Design review of the part built by this model. Coordinates are the model's own, in mm. A direction names the side the tool comes from. Coordinates: 2 decimals unless noted, no trailing zeros. Write each loop counter-clockwise with the first axis right and the second up, starting at its lowest first coordinate (ties: lowest second). Pieces come first, ordered by that corner, then holes. Notation, with made-up numbers: M 52,83 L 58,83 A17 ccw 58,98 Z; hole C -13.5,-20 d4. An arc over 180 degrees is marked long. Return JSON: item names as keys, results as strings. Group by question number.
```python
from build123d import *

# Parameters (mm, degrees)
SKETCH_1_W                   = 110
SKETCH_1_H                   = 42
EXTRUDE_1_DEPTH              = 4
HOLE_WIZARD_M6_1_D           = 5.5
HOLE_WIZARD_M6_1_CBORE_D     = 10
HOLE_WIZARD_M6_1_CBORE_DEPTH = 5.7
HOLE_WIZARD_9_0_9_1_D        = 9
CHAMFER_1_SIZE               = 2
MIRROR_2_COPY_1_D            = 9


with BuildPart() as part:
    # 草图1 → 凸台-拉伸1 (new, symmetric)
    with BuildSketch(Plane(origin=(0, 0, 0), x_dir=(1, 0, 0), z_dir=(0, 1, 0))):
        Rectangle(SKETCH_1_W, SKETCH_1_H)
    extrude(amount=EXTRUDE_1_DEPTH, both=True)

    # M6 六角凹头螺钉的柱形沉头孔1 (through all)
    with Locations(Plane(origin=(0, 4, 0), x_dir=(1, 0, 0), z_dir=(0, 1, 0))):
        with Locations((0, 15), (-12.990381057, -7.5), (12.990381057, -7.5)):
            CounterBoreHole(HOLE_WIZARD_M6_1_D / 2, HOLE_WIZARD_M6_1_CBORE_D / 2, HOLE_WIZARD_M6_1_CBORE_DEPTH)

    # Ø9.0 (9) 直径孔1 (through all)
    with Locations(Plane(origin=(0, -4, 0), x_dir=(-1, 0, 0), z_dir=(0, -1, 0))):
        with Locations((-48, -15)):
            hole_wizard_9_0_9_1 = Hole(HOLE_WIZARD_9_0_9_1_D / 2)

    # 倒角1
    chamfer_1_edges = [part.edges().sort_by_distance(p)[0] for p in [
        (55, 0, 21),
        (-55, 0, 21),
        (-55, 0, -21),
        (55, 0, -21),
    ]]
    chamfer(chamfer_1_edges, length=CHAMFER_1_SIZE)

    # 镜向1: Ø9.0 (9) 直径孔1 across plane
    add(hole_wizard_9_0_9_1.mirror(Plane.XY), mode=Mode.SUBTRACT)

    # 镜向2: Ø9.0 (9) 直径孔1 across plane
    add(hole_wizard_9_0_9_1.mirror(Plane(origin=(0, 0, 0), x_dir=(0, 0, 1), z_dir=(1, 0, 0))), mode=Mode.SUBTRACT)

    # 镜向2 copy 1 (through all)
    with Locations(Plane.XZ.offset(4)):
        with Locations((-48, -15)):
            Hole(MIRROR_2_COPY_1_D / 2)


solid = part.part
```
Item 1: For line 1 (Z direction, x = 48, y = 1.5); line 2 (X direction, y = -3.5, z = -18.5); line 3 (X direction, y = -0.25, z = -16), list the stretches that pass through material, from the lowest coordinate up.
Item 2: The part is to be moulded in two halves that separate along X. For faces 3 (the cylindrical face through (9.305, 1.19, 4.121)), 4 (the flat face through (54, 0, -20)), 5 (the flat face through (-1, -4, 0)), say which applies: pulls with the +X half, pulls with the -X half, needs draft (parallel to the pull), parting line crosses it, or undercut.
Item 3: Add section D-D (x = 48). Write out the cut boundary in (y, z), plus the area to 3 significant figures.
Item 4: For pin 1 (6.5 mm diameter, centred on x = -12.99, z = 7.5, fed in from +Y), flat-tipped, find the tip position at first contact; note if it passes through.
Item 5: Machinability: for faces 1 (the flat face through (2.2, -1.7, -12.8)), 2 (the flat face through (-55, 0, 0)), which of the approach directions +Z, -Z, +X, -X, +Y, -Y give a long, thin tool a straight path to every point of the face, cutting with its end or side? Answer none if there is none.
Item 6: Add section C-C (z = -15). Write out the cut boundary in (x, y).
Item 7: Add section B-B (x = 0). Write out the cut boundary in (y, z), plus the area to 3 significant figures.
Item 8: Add section A-A (z = 15). Write out the cut boundary in (x, y), plus the area to 3 significant figures.
Geometry check:
{
 "1": {"line 1": "-21 to -19.5, -10.5 to 10.5, 19.5 to 21", "line 2": "-55 to -50.83, -45.17 to 45.17, 50.83 to 55", "line 3": "-55 to -52.39, -43.61 to -4.9, 4.9 to 43.61, 52.39 to 55"},
 "2": {"face 3": "undercut", "face 4": "pulls with the +X half", "face 5": "needs draft"},
 "3": {"outline": "M -4,-21 L 4,-21 L 4,-19.5 L -4,-19.5 Z; M -4,-10.5 L 4,-10.5 L 4,10.5 L -4,10.5 Z; M -4,19.5 L 4,19.5 L 4,21 L -4,21 Z", "area": "192 mm^2"},
 "4": {"pin 1": "y = -1.7"},
 "5": {"face 1": "+Y", "face 2": "+Z, -Z, -X, +Y, -Y"},
 "6": {"outline": "M -55,-4 L -52.5,-4 L -52.5,4 L -55,4 Z; M -43.5,-4 L -2.75,-4 L -2.75,-1.7 L -5,-1.7 L -5,4 L -43.5,4 Z; M 2.75,-4 L 43.5,-4 L 43.5,4 L 5,4 L 5,-1.7 L 2.75,-1.7 Z; M 52.5,-4 L 55,-4 L 55,4 L 52.5,4 Z"},
 "7": {"outline": "M -4,-21 L 4,-21 L 4,-20 L -1.7,-20 L -1.7,-17.75 L -4,-17.75 Z; M -4,-12.25 L -1.7,-12.25 L -1.7,-10 L 4,-10 L 4,21 L -4,21 Z", "area": "266 mm^2"},
 "8": {"outline": "M -55,-4 L -52.5,-4 L -52.5,4 L -55,4 Z; M -43.5,-4 L 43.5,-4 L 43.5,4 L -43.5,4 Z; M 52.5,-4 L 55,-4 L 55,4 L 52.5,4 Z", "area": "736 mm^2"}
}
